Model file for the job. Use its own axes, mm. Give positions to 0.01 mm unless a question says otherwise; leave off trailing zeros. Loops run counter-clockwise (first coordinate to the right, second up) from the corner with the lowest first, then second, coordinate; pieces in that order, holes last. Notation, with made-up numbers: (-37, 53) - (8, 53) arc R20 ccw to (8, 57) - close; hole circle Ø5 at (-27, -0.75). An arc over 180 degrees is marked (long way). Use a Markdown table: item, result.
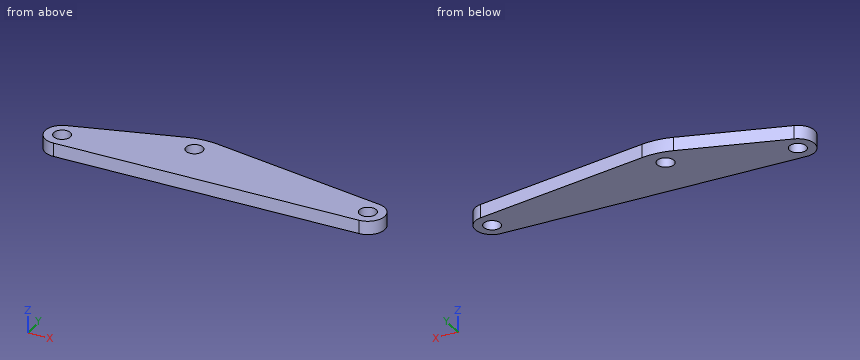
from build123d import *

# Parameters (mm, degrees)
LINK_PROFILE_SKETCH_R = 2.5
LINK_PLATE_4MM_DEPTH  = 4


with BuildPart() as part:
    # Link Profile Sketch → Link Plate 4mm (new body)
    with BuildSketch(Plane.XY):
        with BuildLine():
            Line((52.601773573, 0), (-37.398226427, 0))
            ThreePointArc((-37.398226427, 0), (-42.349566771, 4.304134495), (-38.776413207, 9.80630848))
            Line((-38.776413207, 9.80630848), (-7.835417757, 18.678496156))
            ThreePointArc((-7.835417757, 18.678496156), (-3.369389765, 19.425852932), (1.150292913, 19.149417297))
            Line((1.150292913, 19.149417297), (53.470014461, 9.924038765))
            ThreePointArc((53.470014461, 9.924038765), (57.582747063, 4.564221286), (52.601773573, 0))
        make_face()
        with Locations((-3.085032863, 14)):
            Circle(LINK_PROFILE_SKETCH_R, mode=Mode.SUBTRACT)
        with Locations((-37.398226427, 5)):
            Circle(LINK_PROFILE_SKETCH_R, mode=Mode.SUBTRACT)
        with Locations((52.601773573, 5)):
            Circle(LINK_PROFILE_SKETCH_R, mode=Mode.SUBTRACT)
    extrude(amount=LINK_PLATE_4MM_DEPTH)


solid = part.part
(1) Slice it at A-A, the plane y = 14. Write the cut outline in (x, z), plus the area to 3 significant figures.
Computed:
| item | result |
|---|---|
| outline | (-24.15, 0) - (-5.59, 0) - (-5.59, 4) - (-24.15, 4) - close; (-0.59, 0) - (30.35, 0) - (30.35, 4) - (-0.59, 4) - close |
| area | 198 mm² |
(2) Slice it at B-B, the plane y = 5. Write the cut outline in (x, z).
Computed:
| item | result |
|---|---|
| outline | (-42.4, 0) - (-39.9, 0) - (-39.9, 4) - (-42.4, 4) - close; (-34.9, 0) - (50.1, 0) - (50.1, 4) - (-34.9, 4) - close; (55.1, 0) - (57.6, 0) - (57.6, 4) - (55.1, 4) - close |
(3) Slice it at D-D, the plane x = -10.5. Write the cut outline in (y, z).
Computed:
| item | result |
|---|---|
| outline | (0, 0) - (17.91, 0) - (17.91, 4) - (0, 4) - close |
(4) Slice it at C-C, the plane z = 2.5. Write the cut outline in (x, y).
Computed:
| item | result |
|---|---|
| outline | (-38.78, 9.81) arc R5 ccw to (-37.4, 0) - (52.6, 0) arc R5 ccw to (53.47, 9.92) - (1.15, 19.15) arc R20 ccw to (-7.84, 18.68) - close; hole circle Ø5 at (-37.4, 5); hole circle Ø5 at (-3.09, 14); hole circle Ø5 at (52.6, 5) |
(5) Drill centre lines: probe 1 along X at (y, z) = (4, 3.35); probe 2 along X at (y, z) = (6.25, 2); probe 3 along Y at (x, z) = (53, 0.95). Where is each one in solid material? Low to high. Write a range as [from, to].
Computed:
| item | result |
|---|---|
| probe 1 | [-42.3, -39.69], [-35.11, 50.31], [54.89, 57.5] |
| probe 2 | [-42.24, -39.56], [-35.23, 50.44], [54.77, 57.44] |
| probe 3 | [0.02, 2.53], [7.47, 10.01] |
(6) Pin check, flat tip, straight feed: P1, Ø6.5, axis at x = -37.4, y = 5, coming from the +Z side. Stop position of the tip, or through.
Computed:
| item | result |
|---|---|
| P1 | z = 4 |
